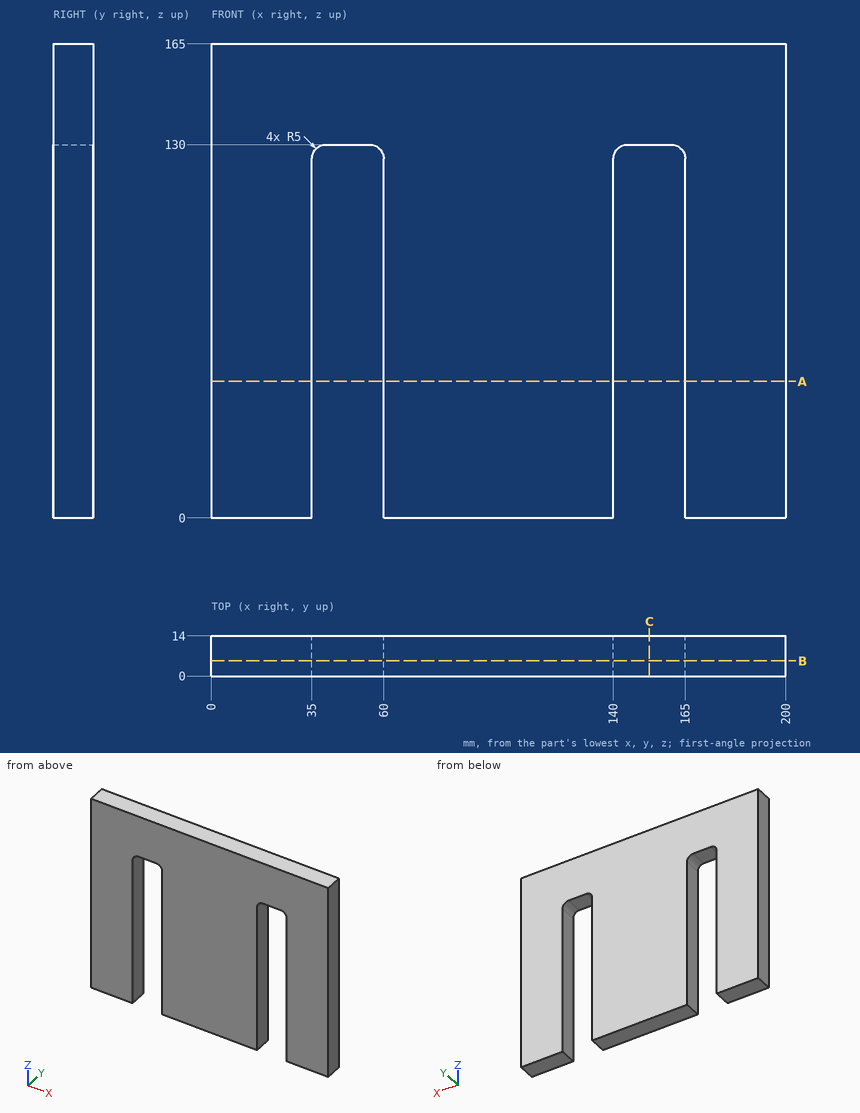
Drawing for the job (mm, zero at the part's lowest x, y, z). Round coordinates to 2 decimals unless told otherwise and drop trailing zeros. Write each loop counter-clockwise with the first axis right and the second up, starting at its lowest first coordinate (ties: lowest second). Pieces come first, ordered by that corner, then holes. Notation, with made-up numbers: M 14,4 L 72,4 A12 ccw 72,12 Z; hole C 20.5,-36.75 d8. An arc over 180 degrees is marked long. Answer as a JSON object with one key per item and string values. Group by question number.
(1) Cut at A-A (z = 47.5). Give the cut face in (x, y), and give its area (3 significant figures).
(2) Drill centre lines: L1, parallel to X at y = 3.5, z = 97.5; L2, parallel to Z at x = 52.5, y = 2.5; L3, parallel to Z at x = 59, y = 2.75. Where is each one in solid material? Low to high.
(3) Cut at B-B (y = 5.25). Give the cut face in (x, z), and give its area (3 significant figures).
(4) Flat gauge pin, fed straight in: pin 1 (7 mm diameter, centred on x = 45, y = 8.5, fed in from -Z). Where does the tip first touch, or does it go through?
(5) Cut at C-C (x = 152.5). Give the cut face in (y, z), and give its area (3 significant figures).
Responses:
{
 "1": {"outline": "M 0,0 L 35,0 L 35,14 L 0,14 Z; M 60,0 L 140,0 L 140,14 L 60,14 Z; M 165,0 L 200,0 L 200,14 L 165,14 Z", "area": "2,100 mm2"},
 "2": {"L1": "x = 0 to 35, 60 to 140, 165 to 200", "L2": "z = 130 to 165", "L3": "z = 128 to 165"},
 "3": {"outline": "M 0,0 L 35,0 L 35,125 A5 cw 40,130 L 55,130 A5 cw 60,125 L 60,0 L 140,0 L 140,125 A5 cw 145,130 L 160,130 A5 cw 165,125 L 165,0 L 200,0 L 200,165 L 0,165 Z", "area": "26,500 mm2"},
 "4": {"pin 1": "stops at z = 130"},
 "5": {"outline": "M 0,130 L 14,130 L 14,165 L 0,165 Z", "area": "490 mm2"}
}
